```python
from build123d import *

# Parameters (mm, degrees)
BASE_PLATE_SKETCH_W     = 100
BASE_PLATE_SKETCH_H     = 60
BASE_PLATE_DEPTH        = 15
UPRIGHT_BLOCK_SKETCH_W  = 50
UPRIGHT_BLOCK_SKETCH_H  = 15
UPRIGHT_BLOCK_DEPTH     = 30
SIDE_WALL_SKETCH_W      = 25.174411278
SIDE_WALL_SKETCH_H      = 15
SIDE_WALL_DEPTH         = 38
LOWER_ARM_SKETCH_W      = 25.174411278
LOWER_ARM_SKETCH_H      = 15
LOWER_ARM_DEPTH         = 45
UPPER_ARM_SKETCH_W      = 15
UPPER_ARM_SKETCH_H      = 15
UPPER_ARM_DEPTH         = 75
WALL_HOLE_SKETCH_R      = 6.5
WALL_THROUGH_HOLE_DEPTH = 75
BASE_HOLE_SKETCH_R      = 10
BASE_THROUGH_HOLE_DEPTH = 75


with BuildPart() as part:
    # Base Plate Sketch → Base Plate (new body)
    with BuildSketch(Plane.XY):
        Rectangle(BASE_PLATE_SKETCH_W, BASE_PLATE_SKETCH_H)
    extrude(amount=BASE_PLATE_DEPTH)

    # Upright Block Sketch → Upright Block (add)
    with BuildSketch(Plane(origin=(0, 0, 0), x_dir=(-1, 0, 0), z_dir=(0, 0, -1))):
        with Locations((-50, -22.5)):
            Rectangle(UPRIGHT_BLOCK_SKETCH_W, UPRIGHT_BLOCK_SKETCH_H)
    extrude(amount=-UPRIGHT_BLOCK_DEPTH)

    # Side Wall Sketch → Side Wall (add)
    with BuildSketch(Plane.XY.offset(30)):
        with Locations((37.587205639, -22.5)):
            Rectangle(SIDE_WALL_SKETCH_W, SIDE_WALL_SKETCH_H)
    extrude(amount=SIDE_WALL_DEPTH)

    # Lower Arm Sketch → Lower Arm (add)
    with BuildSketch(Plane(origin=(0, -15, 0), x_dir=(1, 0, 0), z_dir=(0, 1, 0))):
        with Locations((37.587205639, -60.5)):
            Rectangle(LOWER_ARM_SKETCH_W, LOWER_ARM_SKETCH_H)
    extrude(amount=LOWER_ARM_DEPTH)

    # Upper Arm Sketch → Upper Arm (add)
    with BuildSketch(Plane.ZY.offset(-25)):
        with Locations((60.5, 22.5)):
            Rectangle(UPPER_ARM_SKETCH_W, UPPER_ARM_SKETCH_H)
    extrude(amount=UPPER_ARM_DEPTH)

    # Wall Hole Sketch → Wall Through Hole (cut)
    with BuildSketch(Plane(origin=(0, -15, 0), x_dir=(1, 0, 0), z_dir=(0, 1, 0))):
        with Locations(Location((63, -15, 0), (0, 0, 180))):
            Circle(WALL_HOLE_SKETCH_R)
    extrude(amount=-WALL_THROUGH_HOLE_DEPTH, mode=Mode.SUBTRACT)

    # Base Hole Sketch → Base Through Hole (cut)
    with BuildSketch(Plane.XY.offset(15)):
        Circle(BASE_HOLE_SKETCH_R)
    extrude(amount=-BASE_THROUGH_HOLE_DEPTH, mode=Mode.SUBTRACT)


solid = part.part
```
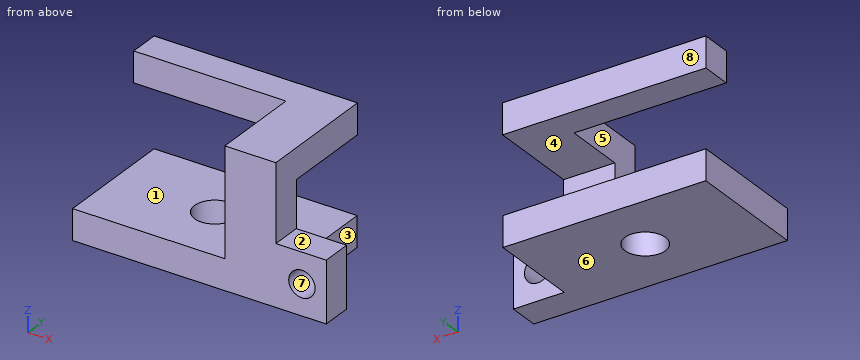
Check sheet for the modelled part. Datum: model origin and axes. Units: mm. Face numbers are marked on the shaded views. A direction names the side the tool comes from. Give positions to 0.01 mm unless a question says otherwise; leave off trailing zeros. Order: outer loops, then holes, each group sorted by start corner. A loop starts at its lowest first (then second) coordinate and runs counter-clockwise, first axis right, second up. Notation, with made-up numbers: (53, 87) -> (71, 87) arc R17 cw to (71, 103) -> close; hole circle Ø2 at (3, 72.25). An arc over 180 degrees is marked (long way). Return JSON: item names as keys, results as strings.
1. Go/stop test with flat-tipped pins: P1, Ø19, axis at y = 13.5, z = 51, coming from the +X side; P2, Ø12, axis at y = -19, z = 35, coming from the -X side; P3, Ø16.5, axis at y = 1, z = 11, coming from the +X side. Record where each tip stops, or that it passes through.
From the geometry:
{"P1": "x = 50.17", "P2": "x = 25", "P3": "x = 50"}
2. Cross-section at D-D, the plane y = -21.5. Record the cut outline in (x, z), plus the area to 3 significant figures.
From the geometry:
{"outline": "(-50, 0) -> (75, 0) -> (75, 30) -> (50.17, 30) -> (50.17, 68) -> (25, 68) -> (25, 15) -> (-50, 15) -> close; hole circle Ø13 at (63, 15)", "area": "3,450 mm^2"}
3. Mould release check, pull along Z, two halves, no side actions. Record for the marked faces 6, 7 and 8: +Z half, -Z half, draft (parallel to the pull), parting line (faces both ways), or undercut.
From the geometry:
{"face 6": "-Z half", "face 7": "undercut", "face 8": "draft"}
4. Material ranges on probe 1 along Z at (x, y) = (63, -19.5); probe 2 along Z at (x, y) = (44, -12); probe 3 along Z at (x, y) = (-32.5, -16), recorded low to high. Write a range as [from, to].
From the geometry:
{"probe 1": "[0, 8.5], [21.5, 30]", "probe 2": "[0, 15], [53, 68]", "probe 3": "[0, 15]"}
5. Cross-section at C-C, the plane z = 7. Record the cut outline in (x, y), plus the area to 3 significant figures.
From the geometry:
{"outline": "(-50, -30) -> (75, -30) -> (75, -15) -> (50, -15) -> (50, 30) -> (-50, 30) -> close; hole circle Ø20 at (0, 0)", "area": "6,060 mm^2"}
6. Cross-section at A-A, the plane x = 0. Record the cut outline in (y, z).
From the geometry:
{"outline": "(-30, 0) -> (-10, 0) -> (-10, 15) -> (-30, 15) -> close; (10, 0) -> (30, 0) -> (30, 15) -> (10, 15) -> close; (15, 53) -> (30, 53) -> (30, 68) -> (15, 68) -> close"}
7. Cross-section at B-B, the plane y = 0. Record the cut outline in (x, z), plus the area to 3 significant figures.
From the geometry:
{"outline": "(-50, 0) -> (-10, 0) -> (-10, 15) -> (-50, 15) -> close; (10, 0) -> (50, 0) -> (50, 15) -> (10, 15) -> close; (25, 53) -> (50.17, 53) -> (50.17, 68) -> (25, 68) -> close", "area": "1,580 mm^2"}
8. Set-up check for the marked faces 1, 2, 3, 4 and 5: record each of +Z, -Z, +X, -X, +Y, -Y from which the full face is reachable in a straight line by a thin tool's end or side.
From the geometry:
{"face 1": "-X, +Y", "face 2": "+Z, +X, +Y, -Y", "face 3": "-Z, +X, +Y", "face 4": "+X, -X, +Y", "face 5": "+Z, -X, -Y"}
